from build123d import *

# Parameters (mm, degrees)
SKETCH1_W           = 40
SKETCH1_H           = 86
BOSS_EXTRUDE1_DEPTH = 6
CHAMFER1_SIZE       = 8.5


with BuildPart() as part:
    # Sketch1 → Boss-Extrude1 (new body)
    with BuildSketch(Plane.XY):
        Rectangle(SKETCH1_W, SKETCH1_H)
    extrude(amount=BOSS_EXTRUDE1_DEPTH)

    # Chamfer1
    chamfer1_edges = [part.edges().sort_by_distance(p)[0] for p in [
        (20, 43, 3),
        (20, -43, 3),
    ]]
    chamfer(chamfer1_edges, length=CHAMFER1_SIZE)


solid = part.part
Build history of the part. All positions in model axes, mm. Round coordinates to 2 decimals unless told otherwise and drop trailing zeros. Write each loop counter-clockwise with the first axis right and the second up, starting at its lowest first coordinate (ties: lowest second). Pieces come first, ordered by that corner, then holes. Notation, with made-up numbers: (89, 74.25) - (136, 74.25) arc R18 cw to (136, 81.25) - close; hole circle Ø7 at (26, -12.5). An arc over 180 degrees is marked (long way). One line per question, with ' | ' between items.
1. Band-saw the part on A-A, the plane z = 3.25. Write the cut outline in (x, y), and give its area (3 significant figures).
Results are:
outline: (-20, -43) - (11.5, -43) - (20, -34.5) - (20, 34.5) - (11.5, 43) - (-20, 43) - close | area: 3,370 mm^2
2. Drill centre lines: line 1 along X through (y, z) = (36, 3.25); line 2 along Y through (x, z) = (14, 1.5); line 3 along Y through (x, z) = (16, 4). Where is each one in solid material? Low to high. Write a range as from..to.
Results are:
line 1: -20..18.5 | line 2: -40.5..40.5 | line 3: -38.5..38.5
3. Band-saw the part on B-B, the plane y = 36.5. Write the cut outline in (x, z), and give its area (3 significant figures).
Results are:
outline: (-20, 0) - (18, 0) - (18, 6) - (-20, 6) - close | area: 228 mm^2
